```python
from build123d import *

# Parameters (mm, degrees)
SHANK_SKETCH_16_R             = 8
SHANK_16X24_DEPTH             = 24
SHANK_END_CHAMFER_0_5X45_SIZE = 0.5
COLLAR_SKETCH_25_R            = 12.5
COLLAR_25X5_DEPTH             = 5
NECK_SKETCH_16_R              = 8
NECK_16X9_DEPTH               = 9
SQUARE_HEAD_SKETCH_16X16_W    = 16
SQUARE_HEAD_SKETCH_16X16_H    = 16
SQUARE_HEAD_16X16X16_DEPTH    = 16


with BuildPart() as part:
    # Shank Sketch Ø16 → Shank Ø16x24 (new body)
    with BuildSketch(Plane(origin=(0, 0, 0), x_dir=(1, 0, 0), z_dir=(0, 1, 0))):
        with Locations(Location((0, 0, 0), (0, 0, 270))):
            Circle(SHANK_SKETCH_16_R)
    extrude(amount=SHANK_16X24_DEPTH)

    # Shank End Chamfer 0.5x45
    shank_end_chamfer_0_5x45_edges = [part.edges().sort_by_distance(p)[0] for p in [
        (0, 0, -8),
    ]]
    chamfer(shank_end_chamfer_0_5x45_edges, length=SHANK_END_CHAMFER_0_5X45_SIZE)

    # Collar Sketch Ø25 → Collar Ø25x5 (add)
    with BuildSketch(Plane(origin=(0, 24, 0), x_dir=(1, 0, 0), z_dir=(0, 1, 0))):
        with Locations(Location((0, 0, 0), (0, 0, 270))):
            Circle(COLLAR_SKETCH_25_R)
    extrude(amount=COLLAR_25X5_DEPTH)

    # Neck Sketch Ø16 → Neck Ø16x9 (add)
    with BuildSketch(Plane(origin=(0, 29, 0), x_dir=(1, 0, 0), z_dir=(0, 1, 0))):
        with Locations(Location((0, 0, 0), (0, 0, 270))):
            Circle(NECK_SKETCH_16_R)
    extrude(amount=NECK_16X9_DEPTH)

    # Square Head Sketch 16x16 → Square Head 16x16x16 (add)
    with BuildSketch(Plane(origin=(0, 38, 0), x_dir=(1, 0, 0), z_dir=(0, 1, 0))):
        Rectangle(SQUARE_HEAD_SKETCH_16X16_W, SQUARE_HEAD_SKETCH_16X16_H)
    extrude(amount=SQUARE_HEAD_16X16X16_DEPTH)


solid = part.part
```
Geometry check sheet. Reference: the model listing, model coordinates, mm. A direction names the side the tool comes from. Coordinates: 2 decimals unless noted, no trailing zeros. Order: outer loops, then holes, each group sorted by start corner. A loop starts at its lowest first (then second) coordinate and runs counter-clockwise, first axis right, second up. Notation, with made-up numbers: (54, -32.5) - (76, -32.5) arc R33 ccw to (76, 3.5) - close; hole circle Ø7 at (85, -0.75). An arc over 180 degrees is marked (long way). Use one line per item in the form item = value.
1. Section check B-B (z = -10.5). Record the boundary of the cut face in (x, y), then the cut area to 3 significant figures.
Here are the results:
outline = (-6.78, 24) - (6.78, 24) - (6.78, 29) - (-6.78, 29) - close
area = 67.8 mm²
2. Gauge pin test, flat ends, axial feed: pin 1 (8 mm diameter, centred on x = 0, z = 8, fed in from -Y); pin 2 (6 mm diameter, centred on x = 4.5, y = 26, fed in from -Z); pin 3 (8 mm diameter, centred on x = 3, y = 14.5, fed in from -Z); pin 4 (5 mm diameter, centred on x = 3, y = 32.5, fed in from +Z). Record the tip position at first contact, or that the pin passes through.
Here are the results:
pin_1 = 0
pin_2 = -12.41
pin_3 = -8
pin_4 = 7.98
3. Section check C-C (y = 48.5). Record the boundary of the cut face in (x, z), then the cut area to 3 significant figures.
Here are the results:
outline = (-8, -8) - (8, -8) - (8, 8) - (-8, 8) - close
area = 256 mm²
4. Draft check along Y on faces 1 (the face through (6, 38, -6)), 2 (the face through (-7.81, 33.44, -1.73)), 3 (the face through (-8.2, 24, -0.2)), 4 (the face through (0, 46, -8)). Enter one of: pulls with the +Y half, pulls with the -Y half, needs draft (parallel to the pull), parting line crosses it, or undercut.
Here are the results:
face_1 = undercut
face_2 = undercut
face_3 = pulls with the -Y half
face_4 = needs draft
5. Access from +Z, -Z, +X, -X, +Y, -Y to the whole of each face (thin tool, end or side, straight path). Record for faces 5 (the face through (0, 46, 8)), 6 (the face through (-6, 38, -6)), 7 (the face through (-8, 46, 0)), 8 (the face through (8, 46, 0)).
Here are the results:
face_5 = +Z, +X, -X, +Y
face_6 = -Z, -X
face_7 = +Z, -Z, -X, +Y
face_8 = +Z, -Z, +X, +Y
6. Section check A-A (y = 30.5). Record the boundary of the cut face in (x, z), then the cut area to 3 significant figures.
Here are the results:
outline = circle Ø16 at (0, 0)
area = 201 mm²
7. Scan lines: line 1 (Y direction, x = -4.25, z = 7.25); line 2 (Z direction, x = -4.25, y = 50.5); line 3 (Y direction, x = 10, z = 0.25). Record each from-to range of solid material in increasing order.
Here are the results:
line_1 = 24 to 29, 38 to 54
line_2 = -8 to 8
line_3 = 24 to 29
